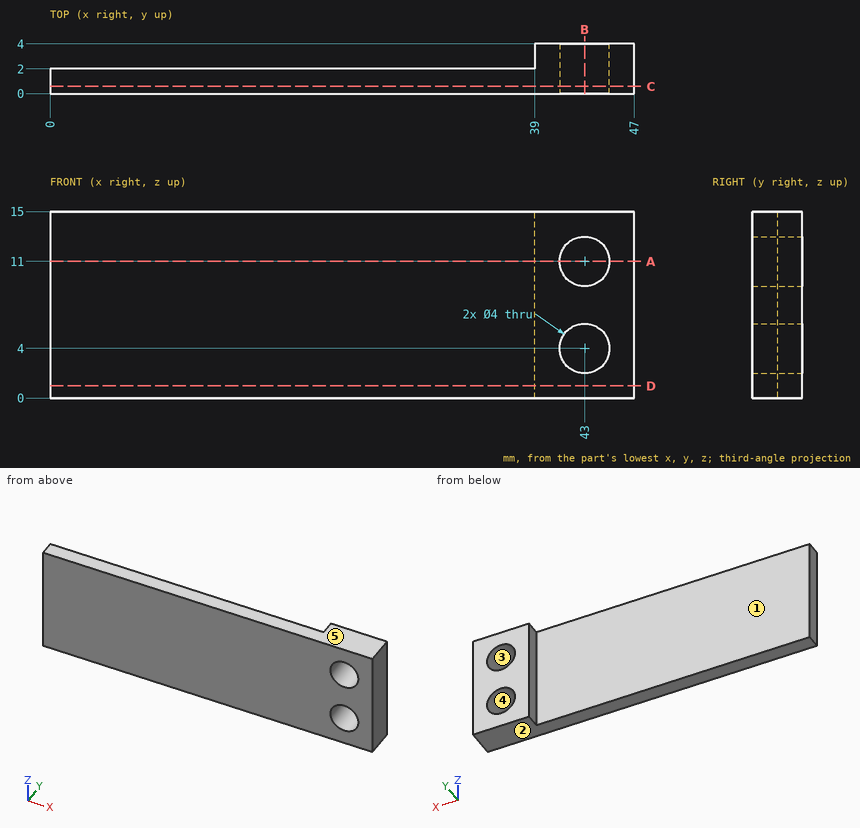
Input: dimensioned drawing with shaded views. Units: mm. Origin: part minimum x, y, z. A direction names the side the tool comes from. Coordinates: 2 decimals unless noted, no trailing zeros. Loops run counter-clockwise (first coordinate to the right, second up) from the corner with the lowest first, then second, coordinate; pieces in that order, holes last. Notation, with made-up numbers: M 80,29 L 99,29 A18 cw 99,44 Z; hole C 11.25,64.25 d5. An arc over 180 degrees is marked long. Use a Markdown table: item, result. Add a question column.
Q1. Material intervals for L1, parallel to Z at x = 43, y = 3.2; L2, parallel to Y at x = 35, z = 3.75; L3, parallel to X at y = 2.85, z = 9.25, sorted ascending.
Q2. Section query C-C, the plane y = 0.6. Return loops of the section in (x, z), and give its area (3 significant figures).
Q3. Section query B-B, the plane x = 43. Return loops of the section in (y, z), and give its area (3 significant figures).
Q4. Draft query along X for the marked faces 3, 4 and 5. Return one class per face: pulls with the +X half, pulls with the -X half, needs draft (parallel to the pull), parting line crosses it, or undercut.
Q5. Section query A-A, the plane z = 11. Return loops of the section in (x, y), and give its area (3 significant figures).
Q6. First-contact query: pin 1 (3 mm diameter, centred on x = 27.5, z = 13, fed in from +Y); pin 2 (1 mm diameter, centred on y = 3.5, z = 8, fed in from -X). Flat tips, straight axial feed; report the tip coordinate or a pass-through.
Q7. Section query D-D, the plane z = 1. Return loops of the section in (x, y), and give its area (3 significant figures).
Q8. Access query for the marked faces 1 and 2. Directions: +Z, -Z, +X, -X, +Y, -Y. A direction counts if a zero-diameter tool reaches every point of the face in a straight line with its end or side. Return the directions, or none.
Result:
| question | item | result |
|---|---|---|
| 1 | L1 | z = 0 to 2, 6 to 9, 13 to 15 |
| 1 | L2 | y = 0 to 2 |
| 1 | L3 | x = 39 to 42.03, 43.97 to 47 |
| 2 | outline | M 0,0 L 47,0 L 47,15 L 0,15 Z; hole C 43,4 d4; hole C 43,11 d4 |
| 2 | area | 680 mm2 |
| 3 | outline | M 0,0 L 4,0 L 4,2 L 0,2 Z; M 0,6 L 4,6 L 4,9 L 0,9 Z; M 0,13 L 4,13 L 4,15 L 0,15 Z |
| 3 | area | 28.0 mm2 |
| 4 | face 3 | undercut |
| 4 | face 4 | undercut |
| 4 | face 5 | needs draft |
| 5 | outline | M 0,0 L 41,0 L 41,4 L 39,4 L 39,2 L 0,2 Z; M 45,0 L 47,0 L 47,4 L 45,4 Z |
| 5 | area | 94.0 mm2 |
| 6 | pin 1 | stops at y = 2 |
| 6 | pin 2 | stops at x = 39 |
| 7 | outline | M 0,0 L 47,0 L 47,4 L 39,4 L 39,2 L 0,2 Z |
| 7 | area | 110 mm2 |
| 8 | face 1 | +Z, -Z, -X, +Y |
| 8 | face 2 | -Z, +X, -X, +Y, -Y |
